Could you check a few things on this drawing? It's one solid part, dimensions in mm from its lowest x, y, z. A direction names the side the tool comes from. Give positions to 0.01 mm unless a question says otherwise; leave off trailing zeros. Loops run counter-clockwise (first coordinate to the right, second up) from the corner with the lowest first, then second, coordinate; pieces in that order, holes last. Notation, with made-up numbers: M 82.5,24 L 138.5,24 A14 cw 138.5,40 Z; hole C 2,-40 d3. An arc over 180 degrees is marked long. Return JSON: item names as keys, results as strings. Group by question number.
1. If we mould it in two halves opening along X, with no side actions, what happens to the marked faces 1 and 2? For each: +X half, -X half, draft (parallel to the pull), parting line (faces both ways), or undercut.
2. If we section it at C-C (y = 111.5): Write out the boundary of the cut face in (x, z).
3. If we section it at A-A (y = 26): Write out the boundary of the cut face in (x, z), plus the area to 3 significant figures.
4. Please list where these lines run through material, in increasing order: line 1 (X direction, y = 85, z = 1.75); line 2 (X direction, y = 17, z = 5); line 3 (Y direction, x = 72.5, z = 6.25).
5. For the marked faces 3, 4, 5, 6 and 7, which set-ups out of +Z, -Z, +X, -X, +Y, -Y let a thin tool reach every point of the face, with its end or its side?
6. If we section it at B-B (z = 2.5): Write out the boundary of the cut face in (x, y).
7. If we section it at D-D (y = 79.5): Write out the boundary of the cut face in (x, z).
8. For pin 1 (4 mm diameter, centred on x = 76, z = 4.5, fed in from -Y); pin 2 (0.8 mm diameter, centred on y = 50.5, z = 13.5, fed in from -X); pin 3 (10 mm diameter, centred on x = 8, y = 64.5, fed in from +Z), each with a flat end and sliding along its axis, tell me the tip position at first contact or that it passes through.
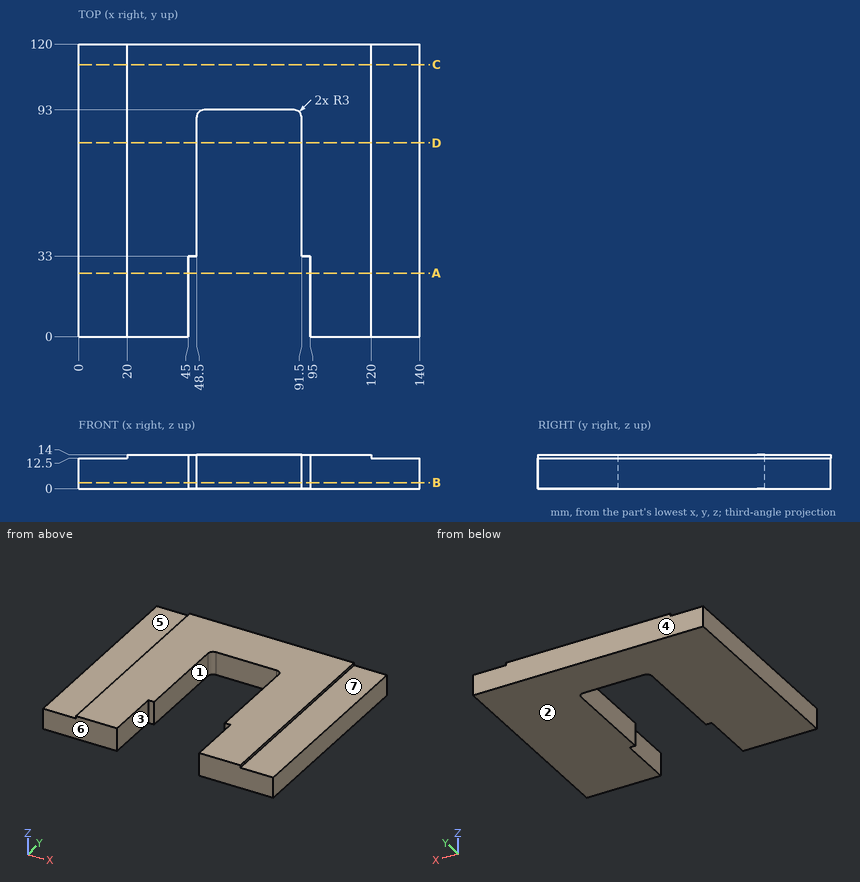
Answer:
{
 "1": {"face 1": "undercut", "face 2": "draft"},
 "2": {"outline": "M 0,0 L 140,0 L 140,12.5 L 120,12.5 L 120,14 L 20,14 L 20,12.5 L 0,12.5 Z"},
 "3": {"outline": "M 0,0 L 45,0 L 45,14 L 20,14 L 20,12.5 L 0,12.5 Z; M 95,0 L 140,0 L 140,12.5 L 120,12.5 L 120,14 L 95,14 Z", "area": "1,200 mm²"},
 "4": {"line 1": "x = 0 to 48.5, 91.5 to 140", "line 2": "x = 0 to 45, 95 to 140", "line 3": "y = 93 to 120"},
 "5": {"face 3": "+Z, -Z, -Y", "face 4": "+Z, -Z, +X, -X, +Y", "face 5": "+Z, -X, +Y, -Y", "face 6": "+Z, -Z, +X, -X, -Y", "face 7": "+Z, +X, +Y, -Y"},
 "6": {"outline": "M 0,0 L 45,0 L 45,33 L 48.5,33 L 48.5,90 A3 cw 51.5,93 L 88.5,93 A3 cw 91.5,90 L 91.5,33 L 95,33 L 95,0 L 140,0 L 140,120 L 0,120 Z"},
 "7": {"outline": "M 0,0 L 48.5,0 L 48.5,14 L 20,14 L 20,12.5 L 0,12.5 Z; M 91.5,0 L 140,0 L 140,12.5 L 120,12.5 L 120,14 L 91.5,14 Z"},
 "8": {"pin 1": "stops at y = 93", "pin 2": "stops at x = 20", "pin 3": "stops at z = 12.5"}
}
